from build123d import *

# Parameters (mm, degrees)
BOSS_EXTRUDE1_DEPTH = 638


with BuildPart() as part:
    # Sketch1 → Boss-Extrude1 (new body)
    with BuildSketch(Plane(origin=(249, 0, 0), x_dir=(0, 0, -1), z_dir=(1, 0, 0))):
        with BuildLine():
            Line((40, -28.571428571), (40, 28.571428571))
            ThreePointArc((40, 28.571428571), (36.652648928, 36.652648928), (28.571428571, 40))
            Line((28.571428571, 40), (-28.571428571, 40))
            ThreePointArc((-28.571428571, 40), (-36.652648928, 36.652648928), (-40, 28.571428571))
            Line((-40, 28.571428571), (-40, -28.571428571))
            ThreePointArc((-40, -28.571428571), (-36.652648928, -36.652648928), (-28.571428571, -40))
            Line((-28.571428571, -40), (28.571428571, -40))
            ThreePointArc((28.571428571, -40), (36.652648928, -36.652648928), (40, -28.571428571))
        make_face()
        with BuildLine():
            Line((-34.285714286, -28.571428571), (-34.285714286, 28.571428571))
            ThreePointArc((-34.285714286, 28.571428571), (-32.61203875, 32.61203875), (-28.571428571, 34.285714286))
            Line((-28.571428571, 34.285714286), (28.571428571, 34.285714286))
            ThreePointArc((28.571428571, 34.285714286), (32.61203875, 32.61203875), (34.285714286, 28.571428571))
            Line((34.285714286, 28.571428571), (34.285714286, -28.571428571))
            ThreePointArc((34.285714286, -28.571428571), (32.61203875, -32.61203875), (28.571428571, -34.285714286))
            Line((28.571428571, -34.285714286), (-28.571428571, -34.285714286))
            ThreePointArc((-28.571428571, -34.285714286), (-32.61203875, -32.61203875), (-34.285714286, -28.571428571))
        make_face(mode=Mode.SUBTRACT)
    extrude(amount=-BOSS_EXTRUDE1_DEPTH)


solid = part.part
The model under review builds one solid part; all positions refer to its coordinate system, in mm. A direction names the side the tool comes from. Coordinates: 2 decimals unless noted, no trailing zeros. Write each loop counter-clockwise with the first axis right and the second up, starting at its lowest first coordinate (ties: lowest second). Pieces come first, ordered by that corner, then holes. Notation, with made-up numbers: (-25.5, 60) - (-14.5, 60) arc R22 cw to (-14.5, 82) - close; hole circle Ø3 at (3, -20.5). An arc over 180 degrees is marked (long way). Answer as CSV lines item,"result".
(1) Mouldability with a two-part tool opening along Z and no side actions: class faces 1 (the flat face through (-389, 1, 36)), 2 (the flat face through (-66, 34.286, 0)), 3 (the cylindrical face through (-65.534, 36.563, -36.741)) as pulls with the +Z half, pulls with the -Z half, needs draft (parallel to the pull), parting line crosses it, or undercut.
Data:
face 1,"needs draft"
face 2,"undercut"
face 3,"pulls with the -Z half"
(2) We need section A-A (x = -116.5). Give the boundary of the cut face in (y, z).
Data:
outline,"(-40, -28.57) arc R11.43 ccw to (-28.57, -40) - (28.57, -40) arc R11.43 ccw to (40, -28.57) - (40, 28.57) arc R11.43 ccw to (28.57, 40) - (-28.57, 40) arc R11.43 ccw to (-40, 28.57) - close; hole (-34.29, -28.57) arc R5.71 ccw to (-28.57, -34.29) - (28.57, -34.29) arc R5.71 ccw to (34.29, -28.57) - (34.29, 28.57) arc R5.71 ccw to (28.57, 34.29) - (-28.57, 34.29) arc R5.71 ccw to (-34.29, 28.57) - close"
(3) Tool access review of faces 4 (the flat face through (-66, 0, 34.286)), 5 (the cylindrical face through (-65.534, -36.563, 36.741)): name each direction out of +Z, -Z, +X, -X, +Y, -Y from which nothing blocks a thin tool from reaching the whole face with its end or side.
Data:
face 4,"+X, -X"
face 5,"+Z, +X, -X, -Y"
(4) We need section B-B (z = -5.5). Give the boundary of the cut face in (x, y).
Data:
outline,"(-389, -40) - (249, -40) - (249, -34.29) - (-389, -34.29) - close; (-389, 34.29) - (249, 34.29) - (249, 40) - (-389, 40) - close"
(5) For line 1 along Y through (x, z) = (208, -19.5); line 2 along Z through (x, y) = (-95.5, 31), list the stretches that pass through material, from the lowest coordinate up. Write a range as [from, to].
Data:
line 1,"y = [-40, -34.29], [34.29, 40]"
line 2,"z = [-39.74, -33.74], [33.74, 39.74]"
